Verification items for the finished model (mm, model axes). A direction names the side the tool comes from. Coordinates: 2 decimals unless noted, no trailing zeros. Write each loop counter-clockwise with the first axis right and the second up, starting at its lowest first coordinate (ties: lowest second). Pieces come first, ordered by that corner, then holes. Notation, with made-up numbers: (-8, 61) -> (19, 61) arc R31 cw to (19, 100) -> close; hole circle Ø10 at (64.5, 37). An arc over 180 degrees is marked (long way). Answer in a Markdown table with one row per item.
```python
from build123d import *

# Parameters (mm, degrees)
BASE_BLOCK_60X135X225_DEPTH = 225
BORE_PROFILE_SKETCH_W       = 72
BORE_PROFILE_SKETCH_H       = 44.5
SECTOR_START                = 17
SECTOR_BOSS_32DEG_X17_DEPTH = 17
END_NOTCH_SKETCH_W          = 20
END_NOTCH_SKETCH_H          = 20
END_NOTCH_20X35_DEPTH       = 97
SLOT_7X95_DEPTH             = 10


with BuildPart() as part:
    # Base Block Sketch → Base Block 60x135x225 (new body)
    with BuildSketch(Plane.XY):
        with BuildLine():
            Line((0, 67.5), (0, 30))
            ThreePointArc((0, 30), (-30, 0), (0, -30))
            Line((0, -30), (0, -67.5))
            ThreePointArc((0, -67.5), (-67.5, 0), (0, 67.5))
        make_face()
    extrude(amount=-BASE_BLOCK_60X135X225_DEPTH)

    # Bore Profile Sketch → Bore Revolve Cut (revolve, cut)
    with BuildSketch(Plane(origin=(0, 0, 0), x_dir=(0, 0, -1), z_dir=(1, 0, 0))):
        with Locations((36, 22.25)):
            Rectangle(BORE_PROFILE_SKETCH_W, BORE_PROFILE_SKETCH_H)
    revolve(axis=Axis((0, 0, 32.736961991), (0, 0, -1)), mode=Mode.SUBTRACT)

    # Sector Boss Sketch → Sector Boss 32deg x17 (add)
    with BuildSketch(Plane.XY.offset(SECTOR_START)):
        with BuildLine():
            Line((-30.348927023, 32.545239722), (-46.034889304, 49.366374859))
            ThreePointArc((-46.034889304, 49.366374859), (-57.858792797, 34.765070056), (-65.199993275, 17.470285544))
            Line((-65.199993275, 17.470285544), (-42.98369927, 11.517447507))
            ThreePointArc((-42.98369927, 11.517447507), (-38.143944881, 22.919194333), (-30.348927023, 32.545239722))
        make_face()
    extrude(amount=-SECTOR_BOSS_32DEG_X17_DEPTH)

    # End Notch Sketch → End Notch 20x35 (cut)
    with BuildSketch(Plane(origin=(0, 0, 0), x_dir=(1, 0, 0), z_dir=(0, 1, 0))):
        with Locations((-10, 180)):
            Rectangle(END_NOTCH_SKETCH_W, END_NOTCH_SKETCH_H)
    extrude(amount=END_NOTCH_20X35_DEPTH, mode=Mode.SUBTRACT)

    # Slot Sketch → Slot 7x95 (cut)
    with BuildSketch(Plane(origin=(0, 0, 0), x_dir=(0, 0, -1), z_dir=(1, 0, 0))):
        with BuildLine():
            Line((239.283215377, -55.75), (130, -55.75))
            ThreePointArc((130, -55.75), (123, -48.75), (130, -41.75))
            Line((130, -41.75), (239.283215377, -41.75))
            ThreePointArc((239.283215377, -41.75), (246.283215377, -48.75), (239.283215377, -55.75))
        make_face()
    extrude(amount=-SLOT_7X95_DEPTH, mode=Mode.SUBTRACT)


solid = part.part
```
1. Sectioned sample at D-D, the plane z = -115. Record the cut outline in (x, y), and give its area (3 significant figures).
Findings below:
| item | result |
|---|---|
| outline | (0, -67.5) -> (0, -30) arc R30 cw to (0, 30) -> (0, 67.5) arc R67.5 ccw to start |
| area | 5,740 mm² |
2. Access from +Z, -Z, +X, -X, +Y, -Y to the whole of each face (thin tool, end or side, straight path). Record for faces 5 (the face through (-23, 50, 0)), 6 (the face through (-20, 43, -180)), 7 (the face through (-5, -55.75, -178)).
Findings below:
| item | result |
|---|---|
| face 5 | +Z, +X, +Y |
| face 6 | +X, +Y |
| face 7 | -Z, +X |
3. Sectioned sample at B-B, the plane y = 27. Record the cut outline in (x, z), and give its area (3 significant figures).
Findings below:
| item | result |
|---|---|
| outline | (-61.86, -225) -> (-13.08, -225) -> (-13.08, -190) -> (-20, -190) -> (-20, -170) -> (-13.08, -170) -> (-13.08, -72) -> (-35.37, -72) -> (-35.37, 17) -> (-61.86, 17) -> close |
| area | 9,680 mm² |
4. Sectioned sample at A-A, the plane z = -161. Record the cut outline in (x, y), and give its area (3 significant figures).
Findings below:
| item | result |
|---|---|
| outline | (-10, -55.75) -> (-10, -41.75) -> (0, -41.75) -> (0, -30) arc R30 cw to (0, 30) -> (0, 67.5) arc R67.5 ccw to (0, -67.5) -> (0, -55.75) -> close |
| area | 5,600 mm² |
5. Sectioned sample at C-C, the plane x = -33. Record the cut outline in (y, z).
Findings below:
| item | result |
|---|---|
| outline | (-58.88, -225) -> (58.88, -225) -> (58.88, 0) -> (35.39, 0) -> (35.39, 17) -> (29.85, 17) -> (29.85, -72) -> (-29.85, -72) -> (-29.85, 0) -> (-58.88, 0) -> close |
6. Go/stop test with flat-tipped pins: pin 1 (10 mm diameter, centred on x = -24.5, z = -194, fed in from -Y); pin 2 (1.5 mm diameter, centred on y = 43.5, z = -97.5, fed in from -X); pin 3 (10.5 mm diameter, centred on x = -20.5, y = 58.5, fed in from +Z). Record where each tip stops, or that it passes through.
Findings below:
| item | result |
|---|---|
| pin 1 | stops at y = -64.62 |
| pin 2 | stops at x = -52.24 |
| pin 3 | stops at z = 0 |
7. Release check for a two-part mould opening along Y. For faces 1 (the face through (-54.247, 14.536, 8.619)), 2 (the face through (-32, 1, -72)), 3 (the face through (-5, -41.75, -177)), 4 (the face through (0, 49, -207)) record: released by +Y, released by -Y, zero draft, split by the parting line, or undercut.
Findings below:
| item | result |
|---|---|
| face 1 | released by -Y |
| face 2 | undercut |
| face 3 | undercut |
| face 4 | zero draft |
8. Material ranges on probe 1 along Y at (x, z) = (-6, -125); probe 2 along Z at (x, y) = (-19.5, -31); probe 3 along Y at (x, z) = (-34.5, -21), recorded low to high. Write a range as from..to.
Findings below:
| item | result |
|---|---|
| probe 1 | y = -67.23..-53.65, -43.85..-29.39, 29.39..67.23 |
| probe 2 | z = -225..-72 |
| probe 3 | y = -58.02..-28.11, 28.11..58.02 |
